Here's how the part is built. I have some questions about the finished solid (model axes, mm). A direction names the side the tool comes from. Round coordinates to 2 decimals unless told otherwise and drop trailing zeros. Order: outer loops, then holes, each group sorted by start corner. A loop starts at its lowest first (then second) coordinate and runs counter-clockwise, first axis right, second up. Notation, with made-up numbers: M -20,-4 L 0,-4 A25 cw 0,15 Z; hole C 51.25,-6 d10. An arc over 180 degrees is marked long. Write item = value, one per line. Start each with the question number.
Item 1: For faces 4 (the face through (100, 49, 10)), 5 (the face through (8, 50, 20)), 6 (the face through (10, 12, 20)), which set-ups out of +Z, -Z, +X, -X, +Y, -Y let a thin tool reach every point of the face, with its end or its side?
Item 2: We'd pull the mould along Y, two halves only. Please class faces 1 (the face through (55, 25, 28)), 2 (the face through (88, 90, 20)), 3 (the face through (49, 0, 10)): pulls with the +Y half, pulls with the -Y half, needs draft (parallel to the pull), parting line crosses it, or undercut.
Item 3: Please list where these lines run through material, in increasing order: L1, parallel to Y at x = 50, z = 21.85; L2, parallel to Z at x = 18.5, y = 22.5; L3, parallel to Z at x = 9.5, y = 89.
Item 4: I want a section at A-A, the plane y = 37.5. List the corners of the cut face in (x, z) for me, plus the area to 3 significant figures.
Item 5: I'm going to push flat-ended pins straight in: P1, Ø12, axis at x = 87.5, y = 48, coming from the -Z side; P2, Ø6, axis at x = 8.5, y = 50, coming from the +Z side; P3, Ø8, axis at x = 9.5, y = 48, coming from the +Z side; P4, Ø5, axis at x = 42.5, z = 26, coming from the +Y side. Where does each tip first touch, or does it pass through?
Item 6: I want a section at D-D, the plane y = 88. List the corners of the cut face in (x, z) for me.
Item 7: I want a section at B-B, the plane x = 29. List the corners of the cut face in (y, z) for me, plus the area to 3 significant figures.
```python
from build123d import *

# Parameters (mm, degrees)
BASE_PLATE_SKETCH_W         = 100
BASE_PLATE_SKETCH_H         = 100
BASE_PLATE_100X100X20_DEPTH = 20
FLANGE_SKETCH_R             = 50
FLANGE_100X5_DEPTH          = 5
FLANGE_BOLT_HOLES_SKETCH_R  = 5
FLANGE_BOLT_HOLES_4X_DEPTH  = 5
HUB_SKETCH_R                = 35
HUB_70X5_DEPTH              = 5
ARC_SLOT_DEPTH              = 5
BORE_SKETCH_R               = 15
BORE_30X5_DEPTH             = 5
ARC_SLOT_PATTERN_3X_COUNT   = 3


with BuildPart() as part:
    # Base Plate Sketch → Base Plate 100x100x20 (new body)
    with BuildSketch(Plane.XY):
        with Locations((50, 50)):
            Rectangle(BASE_PLATE_SKETCH_W, BASE_PLATE_SKETCH_H)
    extrude(amount=BASE_PLATE_100X100X20_DEPTH)

    # Flange Sketch → Flange Ø100x5 (add)
    with BuildSketch(Plane.XY.offset(20)):
        with Locations((50, 50)):
            Circle(FLANGE_SKETCH_R)
    extrude(amount=FLANGE_100X5_DEPTH)

    # Flange Bolt Holes Sketch → Flange Bolt Holes 4x (cut)
    with BuildSketch(Plane.XY.offset(25)):
        with Locations((50, 91.5)):
            Circle(FLANGE_BOLT_HOLES_SKETCH_R)
        with Locations((91.5, 50)):
            Circle(FLANGE_BOLT_HOLES_SKETCH_R)
        with Locations((50, 8.5)):
            Circle(FLANGE_BOLT_HOLES_SKETCH_R)
        with Locations((8.5, 50)):
            Circle(FLANGE_BOLT_HOLES_SKETCH_R)
    extrude(amount=-FLANGE_BOLT_HOLES_4X_DEPTH, mode=Mode.SUBTRACT)

    # Hub Sketch → Hub Ø70x5 (add)
    with BuildSketch(Plane.XY.offset(25)):
        with Locations((50, 50)):
            Circle(HUB_SKETCH_R)
    extrude(amount=HUB_70X5_DEPTH)

    # Arc Slot Sketch → Arc Slot (cut)
    with BuildSketch(Plane.XY.offset(30)):
        with BuildLine():
            ThreePointArc((50, 70), (40, 67.320508076), (32.679491924, 60))
            ThreePointArc((32.679491924, 60), (25.849364905, 58.169872981), (24.019237886, 65))
            ThreePointArc((24.019237886, 65), (35, 75.980762114), (50, 80))
            ThreePointArc((50, 80), (55, 75), (50, 70))
        make_face()
    arc_slot = extrude(amount=-ARC_SLOT_DEPTH, mode=Mode.SUBTRACT)

    # Bore Sketch → Bore Ø30x5 (cut)
    with BuildSketch(Plane.XY.offset(30)):
        with Locations((50, 50)):
            Circle(BORE_SKETCH_R)
    extrude(amount=-BORE_30X5_DEPTH, mode=Mode.SUBTRACT)

    # Arc Slot Pattern 3x: Arc Slot ×3 about axis
    arc_slot_pattern_3x_axis = Axis((50, 50, 0), (0, 0, 1))
    for i in range(1, ARC_SLOT_PATTERN_3X_COUNT):
        add(arc_slot.rotate(arc_slot_pattern_3x_axis, i * 360 / ARC_SLOT_PATTERN_3X_COUNT), mode=Mode.SUBTRACT)


solid = part.part
```
Filled in:
q1.face_4 = +Z, -Z, +X, +Y, -Y
q1.face_5 = +Z
q1.face_6 = +Z, -X, -Y
q2.face_1 = undercut
q2.face_2 = needs draft
q2.face_3 = pulls with the -Y half
q3.L1 = 0 to 3.5, 13.5 to 86.5, 96.5 to 100
q3.L2 = 0 to 25
q3.L3 = 0 to 20
q4.outline = M 0,0 L 100,0 L 100,20 L 98.41,20 L 98.41,25 L 82.69,25 L 82.69,30 L 77.27,30 L 77.27,25 L 66.65,25 L 66.65,30 L 58.29,30 L 58.29,25 L 41.71,25 L 41.71,30 L 34.39,30 L 34.39,25 L 23.35,25 L 23.35,30 L 17.31,30 L 17.31,25 L 1.59,25 L 1.59,20 L 0,20 Z
q4.area = 2,620 mm^2
q5.P1 = 0
q5.P2 = 20
q5.P3 = 25
q5.P4 = 99.73
q6.outline = M 0,0 L 100,0 L 100,20 L 82.5,20 L 82.5,25 L 53.57,25 L 53.57,20 L 46.43,20 L 46.43,25 L 17.5,25 L 17.5,20 L 0,20 Z
q7.outline = M 0,0 L 100,0 L 100,20 L 95.38,20 L 95.38,25 L 78,25 L 78,30 L 71.42,30 L 71.42,25 L 57.54,25 L 57.54,30 L 42.46,30 L 42.46,25 L 28.58,25 L 28.58,30 L 22,30 L 22,25 L 4.62,25 L 4.62,20 L 0,20 Z
q7.area = 2,590 mm^2
